from build123d import *

# Parameters (mm, degrees)
SKETCH1_W            = 615
SKETCH1_H            = 983
BOSS_EXTRUDE1_DEPTH  = 2
SKETCH7_W            = 45
SKETCH7_H            = 91
CUT_EXTRUDE4_DEPTH   = 580.76935069
SKETCH8_R            = 2.25
CUT_EXTRUDE5_DEPTH   = 580.76935069
FILLET3_R            = 10
CUT_EXTRUDE6_DEPTH   = 10
LPATTERN1_COUNT      = 3
LPATTERN1_PITCH      = 431.5
LPATTERN1_COUNT_DIR2 = 2
LPATTERN1_PITCH_DIR2 = 580
SKETCH12_W           = 80
SKETCH12_H           = 150
CUT_EXTRUDE8_DEPTH   = 580.76935069
SKETCH13_W           = 147
SKETCH13_H           = 85
CUT_EXTRUDE9_DEPTH   = 10
FILLET4_R            = 5


with BuildPart() as part:
    # Sketch1 → Boss-Extrude1 (new body)
    with BuildSketch(Plane.XY):
        Rectangle(SKETCH1_W, SKETCH1_H)
    extrude(amount=BOSS_EXTRUDE1_DEPTH)

    # Sketch7 → Cut-Extrude4 (cut, through all)
    with BuildSketch(Plane(origin=(0, 0, 0), x_dir=(-1, 0, 0), z_dir=(0, 0, -1))):
        with Locations((5, 250)):
            Rectangle(SKETCH7_W, SKETCH7_H)
        with Locations((5, -250)):
            Rectangle(SKETCH7_W, SKETCH7_H)
    extrude(amount=-CUT_EXTRUDE4_DEPTH, mode=Mode.SUBTRACT)

    # Sketch8 → Cut-Extrude5 (cut, through all)
    with BuildSketch(Plane(origin=(0, 0, 0), x_dir=(-1, 0, 0), z_dir=(0, 0, -1))):
        with Locations((5, 300)):
            Circle(SKETCH8_R)
        with Locations((5, 200)):
            Circle(SKETCH8_R)
        with Locations((5, -200)):
            Circle(SKETCH8_R)
        with Locations((5, -300)):
            Circle(SKETCH8_R)
    extrude(amount=-CUT_EXTRUDE5_DEPTH, mode=Mode.SUBTRACT)

    # Fillet3
    fillet3_edges = [part.edges().sort_by_distance(p)[0] for p in [
        (307.5, -491.5, 1),
        (-307.5, -491.5, 1),
        (-307.5, 491.5, 1),
        (307.5, 491.5, 1),
    ]]
    fillet(fillet3_edges, radius=FILLET3_R)

    # Sketch10 → Cut-Extrude6 (cut)
    with BuildSketch(Plane(origin=(0, 0, 0), x_dir=(-1, 0, 0), z_dir=(0, 0, -1))):
        with BuildLine():
            Line((292.5, 434.8), (286.9, 434.8))
            ThreePointArc((286.9, 434.8), (277, 431.5), (286.9, 428.2))
            Line((286.9, 428.2), (292.5, 428.2))
            ThreePointArc((292.5, 428.2), (295.8, 431.5), (292.5, 434.8))
        make_face()
    cut_extrude6 = extrude(amount=-CUT_EXTRUDE6_DEPTH, mode=Mode.SUBTRACT)

    # LPattern1: Cut-Extrude6 3 × 2
    with Locations(*[(j * LPATTERN1_PITCH_DIR2, -i * LPATTERN1_PITCH, 0) for i in range(LPATTERN1_COUNT) for j in range(LPATTERN1_COUNT_DIR2) if (i, j) != (0, 0)]):
        add(cut_extrude6, mode=Mode.SUBTRACT)

    # Sketch12 → Cut-Extrude8 (cut, through all)
    with BuildSketch(Plane.XY.offset(2)):
        with Locations((-157.5, -326.5)):
            Rectangle(SKETCH12_W, SKETCH12_H)
    extrude(amount=-CUT_EXTRUDE8_DEPTH, mode=Mode.SUBTRACT)

    # Sketch13 → Cut-Extrude9 (cut)
    with BuildSketch(Plane(origin=(0, 0, 0), x_dir=(-1, 0, 0), z_dir=(0, 0, -1))):
        with Locations((189, -127)):
            Rectangle(SKETCH13_W, SKETCH13_H)
    extrude(amount=-CUT_EXTRUDE9_DEPTH, mode=Mode.SUBTRACT)

    # Fillet4
    fillet4_edges = [part.edges().sort_by_distance(p)[0] for p in [
        (-197.5, -401.5, 1),
        (-197.5, -251.5, 1),
        (-117.5, -251.5, 1),
        (-117.5, -401.5, 1),
        (-115.5, -169.5, 1),
        (-115.5, -84.5, 1),
        (-262.5, -84.5, 1),
        (-262.5, -169.5, 1),
    ]]
    fillet(fillet4_edges, radius=FILLET4_R)


solid = part.part
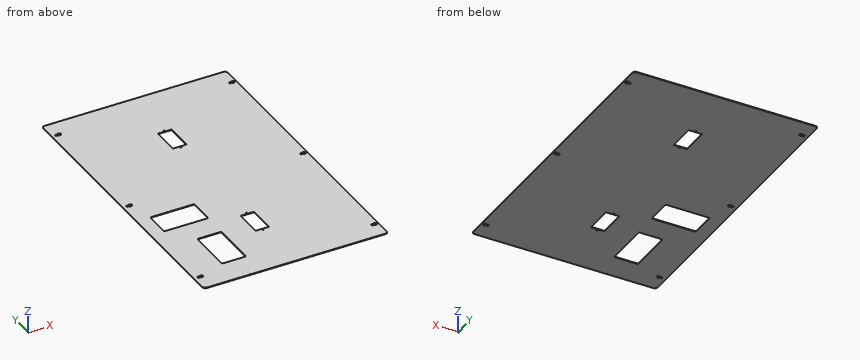
Can you work these out from the model? Positions are in its coordinate system, mm. Coordinates: 2 decimals unless noted, no trailing zeros. Write each loop counter-clockwise with the first axis right and the second up, starting at its lowest first coordinate (ties: lowest second). Pieces come first, ordered by that corner, then holes. Notation, with made-up numbers: (29, -25.5) -> (78, -25.5) arc R22 ccw to (78, 4.5) -> close; hole circle Ø2 at (55, -26). An arc over 180 degrees is marked (long way). Write each question's results on one line, items separated by ' | '. Start each with the question number.
Q1. Imagine slicing it at B-B (x = -235). Write out the boundary of the cut face in (y, z), then the cut area to 3 significant figures.
Q2. Imagine slicing it at D-D (z = 1.35). State how many separate pieces and enclosed holes the cut face has, then the cut area to 3 significant figures.
Q3. If I drill on probe 1 along Y at (x, z) = (-23, 0.55); probe 2 along Y at (x, z) = (297.5, 0.95); probe 3 along X at (y, z) = (0, 1.2), over which ranges is the centre line in solid material (lowest first)?
Q4. Imagine slicing it at A-A (x = -140). Write out the boundary of the cut face in (y, z), then the cut area to 3 significant figures.
Q5. Imagine slicing it at C-C (y = 215.5). Write out the boundary of the cut face in (x, z).
Taken from the geometry:
1) outline: (-491.5, 0) -> (-169.5, 0) -> (-169.5, 2) -> (-491.5, 2) -> close; (-84.5, 0) -> (491.5, 0) -> (491.5, 2) -> (-84.5, 2) -> close | area: 1,800 mm^2
2) separate pieces: 1 | enclosed holes: 14 | area: 571,000 mm^2
3) probe 1: y = -491.5 to -295.5, -204.5 to 204.5, 295.5 to 491.5 | probe 2: y = -491.5 to -437, -426 to -5.5, 5.5 to 426, 437 to 491.5 | probe 3: x = -307.5 to -295.8, -277 to 284.2, 303 to 307.5
4) outline: (-491.5, 0) -> (-401.5, 0) -> (-401.5, 2) -> (-491.5, 2) -> close; (-251.5, 0) -> (-169.5, 0) -> (-169.5, 2) -> (-251.5, 2) -> close; (-84.5, 0) -> (491.5, 0) -> (491.5, 2) -> (-84.5, 2) -> close | area: 1,500 mm^2
5) outline: (-307.5, 0) -> (-27.5, 0) -> (-27.5, 2) -> (-307.5, 2) -> close; (17.5, 0) -> (307.5, 0) -> (307.5, 2) -> (17.5, 2) -> close
